Read the model definition and answer for the solid it produces. Units are mm, in the model's axes. A direction names the side the tool comes from. Coordinates: 2 decimals unless noted, no trailing zeros. Loops run counter-clockwise (first coordinate to the right, second up) from the corner with the lowest first, then second, coordinate; pieces in that order, holes last.
from build123d import *

# Parameters (mm, degrees)
FLANGE_PLATE_DEPTH     = 15
SIDE_NOTCH_SKETCH_R    = 5
SIDE_NOTCH_10X10_DEPTH = 15
HUB_BOSS_SKETCH_R      = 20
HUB_BOSS_40_DEPTH      = 15
BORE_SKETCH_R          = 10
BORE_20_DEPTH          = 15


with BuildPart() as part:
    # Flange Plate Profile Sketch → Flange Plate (new body)
    with BuildSketch(Plane.XY):
        with BuildLine():
            Line((9.999999107, -5.133e-06), (59.999999107, -5.133e-06))
            ThreePointArc((59.999999107, -5.133e-06), (69.999996541, 10), (79.999999107, 0))
            Line((79.999999107, 0), (79.999999107, -50))
            ThreePointArc((79.999999107, -50), (70.000001674, -60), (59.999999107, -50.000005133))
            Line((59.999999107, -50.000005133), (10.000000893, -50.000005133))
            ThreePointArc((10.000000893, -50.000005133), (1.674e-06, -60.000006696), (-9.999999107, -50.000006696))
            Line((-9.999999107, -50.000006696), (-9.999999107, -30))
            Line((-9.999999107, -30), (5.000000893, -30))
            ThreePointArc((5.000000893, -30), (10.000001691, -25.000000893), (5.000002678, -20))
            Line((5.000002678, -20), (-9.999999107, -20))
            Line((-9.999999107, -20), (-9.999999107, 0))
            ThreePointArc((-9.999999107, 0), (2.567e-06, 9.999999107), (9.999999107, -5.133e-06))
        make_face()
    extrude(amount=FLANGE_PLATE_DEPTH)

    # Side Notch Sketch → Side Notch 10x10 (cut)
    with BuildSketch(Plane.XY.offset(15)):
        Circle(SIDE_NOTCH_SKETCH_R)
        with Locations((69.999999107, 0)):
            Circle(SIDE_NOTCH_SKETCH_R)
        with Locations((69.999999107, -50)):
            Circle(SIDE_NOTCH_SKETCH_R)
        with Locations((8.93e-07, -50.000006696)):
            Circle(SIDE_NOTCH_SKETCH_R)
    extrude(amount=-SIDE_NOTCH_10X10_DEPTH, mode=Mode.SUBTRACT)

    # Hub Boss Sketch → Hub Boss Ø40 (add)
    with BuildSketch(Plane.XY.offset(15)):
        with Locations((34.999999107, -25.000005133)):
            Circle(HUB_BOSS_SKETCH_R)
    extrude(amount=HUB_BOSS_40_DEPTH)

    # Bore Sketch → Bore Ø20 (cut)
    with BuildSketch(Plane.XY.offset(30)):
        with Locations((34.999999107, -25.000005133)):
            Circle(BORE_SKETCH_R)
    extrude(amount=-BORE_20_DEPTH, mode=Mode.SUBTRACT)


solid = part.part
Item 1: Given pin 1 (3 mm diameter, centred on x = 19.5, z = 11, fed in from -Y); pin 2 (3 mm diameter, centred on x = 53.5, z = 8, fed in from +Y); pin 3 (8 mm diameter, centred on x = 44.5, z = 25.5, fed in from +Y); pin 4 (6 mm diameter, centred on x = 70, y = 0, fed in from -Z), each flat-ended and moving along its own axis, determine where each tip first touches the part or whether it passes through.
Numbers:
pin 1: stops at y = -50
pin 2: stops at y = 0
pin 3: stops at y = -5.77
pin 4: passes through
Item 2: Determine the mould class of faces 3 (the face through (35, 0, 7)), 4 (the face through (36, -25, 0)), 5 (the face through (-1.08, -54.88, 7.6)), 6 (the face through (0, -60, 7)) for opening direction Y: released by +Y, released by -Y, zero draft, split by the parting line, or undercut.
Numbers:
face 3: released by +Y
face 4: zero draft
face 5: undercut
face 6: released by -Y
Item 3: Find the intervals of material crossed by line 1 along Y through (x, z) = (0, 10.75); line 2 along Y through (x, z) = (70, 3.75); line 3 along X through (y, z) = (-2.5, 3), in increasing order.
Numbers:
line 1: y = -60 to -55, -45 to -30, -20 to -5, 5 to 10
line 2: y = -60 to -55, -45 to -5, 5 to 10
line 3: x = -10 to -4.33, 4.33 to 65.67, 74.33 to 80
Item 4: A cutting plane is placed at A-A on y = -47. Determine the outline of the cut face in (x, z).
Numbers:
outline: (-10, 0) - (-4, 0) - (-4, 15) - (-10, 15) - close; (4, 0) - (66, 0) - (66, 15) - (4, 15) - close; (74, 0) - (80, 0) - (80, 15) - (74, 15) - close
Item 5: A cutting plane is placed at B-B on x = 70. Determine the outline of the cut face in (y, z), then the cut area to 3 significant figures.
Numbers:
outline: (-60, 0) - (-55, 0) - (-55, 15) - (-60, 15) - close; (-45, 0) - (-5, 0) - (-5, 15) - (-45, 15) - close; (5, 0) - (10, 0) - (10, 15) - (5, 15) - close
area: 750 mm2
Item 6: A cutting plane is placed at C-C on z = 12. Determine the outline of the cut face in (x, y).
Numbers:
outline: (-10, -50) arc R10 ccw to (10, -50) - (60, -50) arc R10 ccw to (80, -50) - (80, 0) arc R10 ccw to (60, 0) - (10, 0) arc R10 ccw to (-10, 0) - (-10, -20) - (5, -20) arc R5 cw to (5, -30) - (-10, -30) - close; hole circle Ø10 at (0, -50); hole circle Ø10 at (0, 0); hole circle Ø10 at (70, -50); hole circle Ø10 at (70, 0)
Item 7: A cutting plane is placed at D-D on x = 6. Determine the outline of the cut face in (y, z).
Numbers:
outline: (-58, 0) - (-29.9, 0) - (-29.9, 15) - (-58, 15) - close; (-20.1, 0) - (8, 0) - (8, 15) - (-20.1, 15) - close
Item 8: Which of the six approach directions +Z, -Z, +X, -X, +Y, -Y give full straight-line access (tool end or side, diameter ignored) to faces 1 (the face through (27, -31, 23)), 2 (the face through (-1.08, -4.88, 7.6))?
Numbers:
face 1: +Z
face 2: +Z, -Z
